For this review, take the finished solid that the model builds, in its own axes (mm). Face numbers are marked on the shaded views. A direction names the side the tool comes from. Give positions to 0.01 mm unless a question says otherwise; leave off trailing zeros. Order: outer loops, then holes, each group sorted by start corner. A loop starts at its lowest first (then second) coordinate and runs counter-clockwise, first axis right, second up. Notation, with made-up numbers: M 58.5,-1.75 L 107.5,-1.75 A16 cw 107.5,7.25 Z; hole C -36,-12.5 d10. An arc over 180 degrees is marked long. Use CSV: the item, a comma, the result in double quotes. Start each with the question number.
(1) Consider section C-C (z = -2). Write out the cut boundary in (x, y).
(2) Draft analysis for pull direction Z (two halves, no side actions). For the marked faces 4, 5 and 6, state which applies: pulls with the +Z half, pulls with the -Z half, needs draft (parallel to the pull), parting line crosses it, or undercut.
(3) Clearance check with flat-ended pins moving along their axes: P1, Ø6, axis at x = 2, y = -4, coming from the +Z side; P2, Ø1.2, axis at y = 0, z = -2, coming from the +X side; P3, Ø3, axis at y = 0, z = -2, coming from the +X side; P4, Ø2, axis at x = -4.5, z = 1.5, coming from the +Y side. State where each tip first meets the part, or that it passes through.
(4) Tool access review of the marked faces 1, 2 and 3: name each direction out of +Z, -Z, +X, -X, +Y, -Y from which nothing blocks a thin tool from reaching the whole face with its end or side.
(5) Wall thickness on L1, parallel to Y at x = 0, z = -0.75; L2, parallel to Y at x = 0, z = 1.25; L3, parallel to Z at x = -3.6, y = 0: over which ranges is each line inside the solid? List them lowest first. Write a range as from..to.
(6) Consider section B-B (y = 0). Write out the cut boundary in (x, z).
(7) Consider section D-D (z = -0.75). Write out the cut boundary in (x, y).
(8) Consider section A-A (x = 0). Write out the cut boundary in (y, z).
```python
from build123d import *

# Parameters (mm, degrees)
SKETCH1_R           = 10
BOSS_EXTRUDE1_DEPTH = 3
SKETCH2_R           = 2.5
BOSS_EXTRUDE2_DEPTH = 3
SKETCH3_R           = 1.5
BOSS_EXTRUDE3_DEPTH = 2
SKETCH4_R           = 3
CUT_EXTRUDE1_DEPTH  = 24
BOSS_EXTRUDE4_START = 4
SKETCH5_R           = 4
SKETCH5_R_2         = 3
BOSS_EXTRUDE4_DEPTH = 4
SKETCH6_R           = 1
CUT_EXTRUDE2_DEPTH  = 5


with BuildPart() as part:
    # Sketch1 → Boss-Extrude1 (new body)
    with BuildSketch(Plane.XY):
        Circle(SKETCH1_R)
    extrude(amount=BOSS_EXTRUDE1_DEPTH)

    # Sketch2 → Boss-Extrude2 (add)
    with BuildSketch(Plane.XY.offset(3)):
        with Locations((0, 7)):
            Circle(SKETCH2_R)
    extrude(amount=BOSS_EXTRUDE2_DEPTH)

    # Sketch3 → Boss-Extrude3 (add)
    with BuildSketch(Plane.XY.offset(6)):
        with Locations((0, 7)):
            Circle(SKETCH3_R)
    extrude(amount=BOSS_EXTRUDE3_DEPTH)

    # Sketch4 → Cut-Extrude1 (cut)
    with BuildSketch(Plane(origin=(0, 0, 0), x_dir=(-1, 0, 0), z_dir=(0, 0, -1))):
        Circle(SKETCH4_R)
    extrude(amount=-CUT_EXTRUDE1_DEPTH, mode=Mode.SUBTRACT)

    # Sketch5 → Boss-Extrude4 (add)
    with BuildSketch(Plane(origin=(0, 0, 0), x_dir=(-1, 0, 0), z_dir=(0, 0, -1)).offset(BOSS_EXTRUDE4_START)):
        with Locations(Location((0, 0, 0), (0, 0, 180))):
            Circle(SKETCH5_R)
        Circle(SKETCH5_R_2, mode=Mode.SUBTRACT)
    extrude(amount=-BOSS_EXTRUDE4_DEPTH)

    # Sketch6 → Cut-Extrude2 (cut, symmetric)
    with BuildSketch(Plane(origin=(0, 0, 0), x_dir=(0, 0, -1), z_dir=(1, 0, 0))):
        with Locations((2, 0)):
            Circle(SKETCH6_R)
    extrude(amount=CUT_EXTRUDE2_DEPTH, both=True, mode=Mode.SUBTRACT)


solid = part.part
```
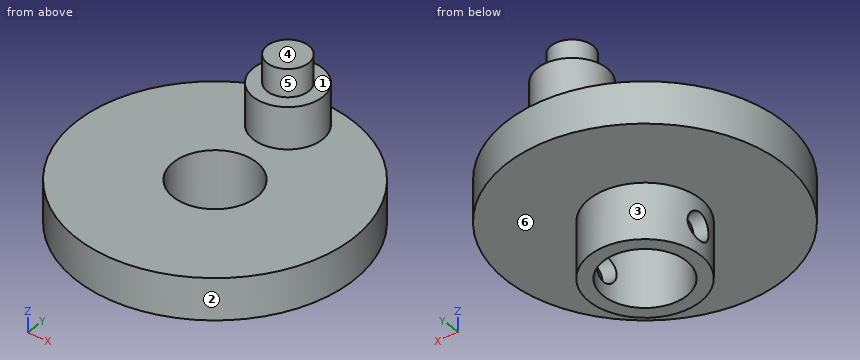
Check result:
1,outline,"M -3.87,-1 A4 ccw 3.87,-1 L 2.83,-1 A3 cw -2.83,-1 Z; M -3.87,1 L -2.83,1 A3 cw 2.83,1 L 3.87,1 A4 ccw Z"
2,face 4,"pulls with the +Z half"
2,face 5,"needs draft"
2,face 6,"pulls with the -Z half"
3,P1,"stops at z = 3"
3,P2,"passes through"
3,P3,"stops at x = 4"
3,P4,"stops at y = 9.37"
4,face 1,"+Z"
4,face 2,"+Z, -Z"
4,face 3,"-Z"
5,L1,"y = -4..-3, 3..4"
5,L2,"y = -10..-3, 3..10"
5,L3,"z = -4..-3, -1..3"
6,outline,"M -10,0 L -4,0 L -4,-1 L -3,-1 L -3,3 L -10,3 Z; M -4,-4 L -3,-4 L -3,-3 L -4,-3 Z; M 3,-4 L 4,-4 L 4,-3 L 3,-3 Z; M 3,-1 L 4,-1 L 4,0 L 10,0 L 10,3 L 3,3 Z"
7,outline,"C 0,0 d8; hole C 0,0 d6"
8,outline,"M -10,0 L -4,0 L -4,-4 L -3,-4 L -3,3 L -10,3 Z; M 3,-4 L 4,-4 L 4,0 L 10,0 L 10,3 L 9.5,3 L 9.5,6 L 8.5,6 L 8.5,8 L 5.5,8 L 5.5,6 L 4.5,6 L 4.5,3 L 3,3 Z"
